Work out the finished part from the listing and answer in its coordinate system (mm). Give positions to 0.01 mm unless a question says otherwise; leave off trailing zeros. Loops run counter-clockwise (first coordinate to the right, second up) from the corner with the lowest first, then second, coordinate; pieces in that order, holes last.
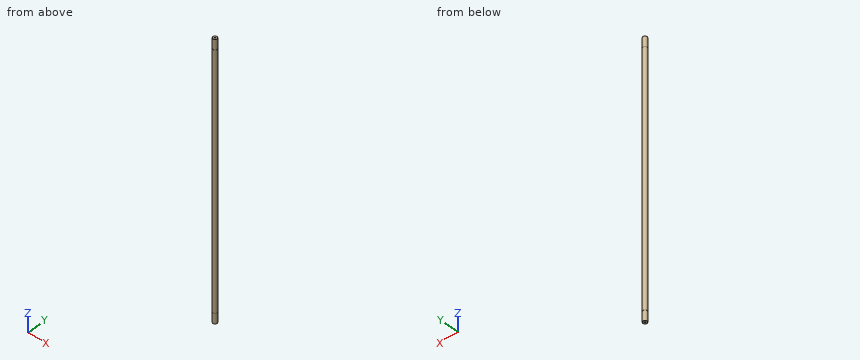
from build123d import *

# Parameters (mm, degrees)
SKETCH_1_R      = 12.5
EXTRUDE_1_DEPTH = 1600
CHAMFER_1_SIZE  = 0.5
SKETCH_2_W      = 0.55
SKETCH_2_H      = 1.3


with BuildPart() as part:
    # 草图1 → 凸台-拉伸1 (new body)
    with BuildSketch(Plane.XY):
        Circle(SKETCH_1_R)
    extrude(amount=EXTRUDE_1_DEPTH)

    # 倒角1
    chamfer_1_edges = [part.edges().sort_by_distance(p)[0] for p in [
        (-12.5, 0, 0),
        (-12.5, 0, 1600),
    ]]
    chamfer(chamfer_1_edges, length=CHAMFER_1_SIZE)

    # 草图2 → 切除-旋转1 (revolve, cut)
    with BuildSketch(Plane(origin=(0, 0, 0), x_dir=(1, 0, 0), z_dir=(0, 1, 0))):
        with Locations((12.225, -1540.55)):
            Rectangle(SKETCH_2_W, SKETCH_2_H)
    cut_revolve_1 = revolve(axis=Axis((0, 0, 1599.5), (0, 0, -1)), mode=Mode.SUBTRACT)

    # 草图5 → M8 螺纹孔1 (revolve, cut)
    with BuildSketch(Plane(origin=(0, 0, 1600), x_dir=(0, -1, 0), z_dir=(1, 0, 0))):
        Polygon((0, 0), (0, 21.792926105), (3.4, 19.75), (3.4, 0), align=None)
    hole_wizard_m8_1 = revolve(axis=Axis((0, 0, 1606.35), (0, 0, -1)), mode=Mode.SUBTRACT)

    # 镜向1: 切除-旋转1, M8 螺纹孔1 across plane
    add(cut_revolve_1.mirror(Plane.XY.offset(800)), mode=Mode.SUBTRACT)
    add(hole_wizard_m8_1.mirror(Plane.XY.offset(800)), mode=Mode.SUBTRACT)


solid = part.part
Item 1: Consider line 1 (Y direction, x = 0, z = 1591); line 2 (Z direction, x = -6.5, y = 10.25). Determine where each line is inside the solid, lowest interval first.
Item 2: Flat-ended cylindrical pins translate along their axes: pin 1 Ø1.5 at (y, z) = (9.5, 1209) entering from -X; pin 2 Ø2 at (x, z) = (9, 1184.5) entering from -Y; pin 3 Ø2 at (y, z) = (-8.5, 827) entering from -X. Find the tip coordinate at first contact, or state that the pin passes through.
Item 3: Find section A-A, the plane z = 181. Write down the section's boundary in (x, y).
Ans:
1. line 1: y = -12.5 to -3.4, 3.4 to 12.5
1. line 2: z = 0.14 to 58.8, 60.1 to 1539.9, 1541.2 to 1599.86
2. pin 1: stops at x = -8.93
2. pin 2: stops at y = -9.6
2. pin 3: stops at x = -10
3. outline: circle Ø25 at (0, 0)
